from build123d import *

# Parameters (mm, degrees)
HEX_HEAD_5AF_X_3_DEPTH = 3
SHANK_PROFILE_3_R      = 1.5
SHANK_3_X_10_DEPTH     = 10


with BuildPart() as part:
    # Hex Head Profile → Hex Head 5AF x 3 (new body)
    with BuildSketch(Plane(origin=(0, 0, 0), x_dir=(1, 0, 0), z_dir=(0, 1, 0))):
        Polygon((2.886751346, 0), (1.443375673, 2.5), (-1.443375673, 2.5), (-2.886751346, 0), (-1.443375673, -2.5), (1.443375673, -2.5), align=None)
    extrude(amount=HEX_HEAD_5AF_X_3_DEPTH)

    # Shank Profile Ø3 → Shank Ø3 x 10 (add)
    with BuildSketch(Plane.XZ):
        with Locations(Location((0, 0, 0), (0, 0, 270))):
            Circle(SHANK_PROFILE_3_R)
    extrude(amount=SHANK_3_X_10_DEPTH)


solid = part.part
Part model, mm, in its own coordinate system. A direction names the side the tool comes from. Give positions to 0.01 mm unless a question says otherwise; leave off trailing zeros. Loops run counter-clockwise (first coordinate to the right, second up) from the corner with the lowest first, then second, coordinate; pieces in that order, holes last. Notation, with made-up numbers: (81.5, -35.5) -> (105.5, -35.5) arc R11 cw to (105.5, -16.5) -> close; hole circle Ø10 at (-14, -13.75). An arc over 180 degrees is marked (long way). Write each question's results on one line, items separated by ' | '. Start each with the question number.
Q1. Band-saw the part on C-C on z = -0.8. List the corners of the cut face in (x, y).
Q2. Band-saw the part on A-A on x = 0. List the corners of the cut face in (y, z), plus the area to 3 significant figures.
Q3. Band-saw the part on B-B on y = 2.25. List the corners of the cut face in (x, z).
Q4. Pin check, flat tips, straight feed: P1, Ø1.5, axis at x = -1.5, y = -5, coming from the +Z side; P2, Ø1, axis at x = 0, y = -2, coming from the +Z side; P3, Ø1, axis at y = -5.5, z = -1, coming from the +X side. Stop position of each tip, or through.
Q5. Which spindle directions (+Z, -Z, +X, -X, +Y, -Y) get a long thin tool onto all of the face, cutting with end or side? Do faces 1 (the face through (1.24, 0, -1.15)), 2 (the face through (0, -10, 0)). Say none if no direction does.
Q6. Band-saw the part on D-D on y = -6.25. List the corners of the cut face in (x, z).
Q7. Wall check: L1, parallel to Y at x = -0.95, z = -1.2; L2, parallel to Z at x = -0.55, y = -1; L3, parallel to X at y = -1.25, z = -0.45. Give the ranges that are in metal, low to high.
Results are:
1) outline: (-2.42, 0) -> (-1.27, 0) -> (-1.27, -10) -> (1.27, -10) -> (1.27, 0) -> (2.42, 0) -> (2.42, 3) -> (-2.42, 3) -> close
2) outline: (-10, -1.5) -> (0, -1.5) -> (0, -2.5) -> (3, -2.5) -> (3, 2.5) -> (0, 2.5) -> (0, 1.5) -> (-10, 1.5) -> close | area: 45.0 mm²
3) outline: (-2.89, 0) -> (-1.44, -2.5) -> (1.44, -2.5) -> (2.89, 0) -> (1.44, 2.5) -> (-1.44, 2.5) -> close
4) P1: stops at z = 1.3 | P2: stops at z = 1.5 | P3: stops at x = 1.41
5) face 1: -Y | face 2: +Z, -Z, +X, -X, -Y
6) outline: circle Ø3 at (0, 0)
7) L1: y = 0 to 3 | L2: z = -1.4 to 1.4 | L3: x = -1.43 to 1.43
